Model file for the job. Use its own axes, mm. Face numbers are marked on the shaded views. A direction names the side the tool comes from. Round coordinates to 2 decimals unless told otherwise and drop trailing zeros. Loops run counter-clockwise (first coordinate to the right, second up) from the corner with the lowest first, then second, coordinate; pieces in that order, holes last. Notation, with made-up numbers: M 24,18.25 L 82,18.25 A14 cw 82,37.25 Z; hole C 61.25,35 d11. An arc over 180 degrees is marked long. Answer in a Markdown table with one row per item.
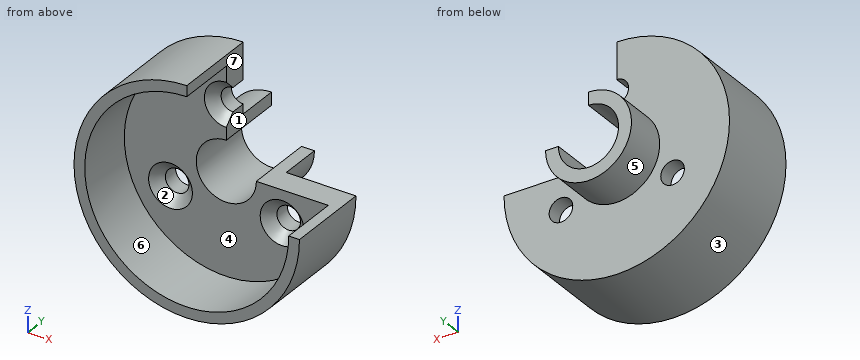
from build123d import *

# Parameters (mm, degrees)
COUNTERSUNK_HOLE_11_D             = 11
COUNTERSUNK_HOLE_11_CSINK_D       = 20.4
COUNTERSUNK_HOLE_11_CSINK_ANGLE   = 90
COUNTERSUNK_HOLE_PATTERN_3X_COUNT = 3
SIDE_SLOT_CUT_DEPTH               = 81.848623983
SIDE_SLOT_CUT_DEPTH_BACK          = 81.848623983


with BuildPart() as part:
    # Bed Profile Sketch → Bed Body Revolve (revolve)
    with BuildSketch(Plane(origin=(0, 0, 0), x_dir=(0, 0, -1), z_dir=(1, 0, 0))):
        Polygon((14, 30.393677345), (14, -1.606322655), (47.5, -1.606322655), (47.5, -29.606322655), (52.5, -29.606322655), (52.5, 10.393677345), (20, 10.393677345), (20, 30.393677345), align=None)
    revolve(axis=Axis((0, 0, 0), (0, 1, 0)))

    # Countersunk Hole Ø11 (through all)
    with Locations(Plane(origin=(0, -1.606322655, 30), x_dir=(0, 0, -1), z_dir=(0, -1, 0))):
        with Locations((0, 0)):
            countersunk_hole_11 = CounterSinkHole(COUNTERSUNK_HOLE_11_D / 2, COUNTERSUNK_HOLE_11_CSINK_D / 2, counter_sink_angle=COUNTERSUNK_HOLE_11_CSINK_ANGLE)

    # Countersunk Hole Pattern 3x: Countersunk Hole Ø11 ×3 about axis
    countersunk_hole_pattern_3x_axis = Axis((0, 0, 0), (0, 1, 0))
    for i in range(1, COUNTERSUNK_HOLE_PATTERN_3X_COUNT):
        add(countersunk_hole_11.rotate(countersunk_hole_pattern_3x_axis, i * 360 / COUNTERSUNK_HOLE_PATTERN_3X_COUNT), mode=Mode.SUBTRACT)

    # Side Slot Sketch → Side Slot Cut (cut, two sides: drawn at the far end of the back side and taken through both)
    with BuildSketch(Plane.XZ.offset(1.606322655).offset(-SIDE_SLOT_CUT_DEPTH_BACK)):
        with BuildLine():
            Line((0, 66.315052509), (0, 0))
            Line((0, 0), (70.372177226, 0))
            ThreePointArc((70.372177226, 0), (52.403266899, 51.428043669), (0, 66.315052509))
        make_face()
    extrude(amount=SIDE_SLOT_CUT_DEPTH + SIDE_SLOT_CUT_DEPTH_BACK, mode=Mode.SUBTRACT)


solid = part.part
1. Pin check, flat tips, straight feed: pin 1 (1 mm diameter, centred on x = 3.5, y = -16, fed in from +Z); pin 2 (4 mm diameter, centred on x = -36.5, z = 36, fed in from +Y); pin 3 (5 mm diameter, centred on x = -20, z = -37.5, fed in from -Y); pin 4 (9 mm diameter, centred on x = 25.98, z = -15, fed in from +Y). Stop position of each tip, or through.
Verdict:
| item | result |
|---|---|
| pin 1 | stops at z = -47.33 |
| pin 2 | stops at y = 10.39 |
| pin 3 | stops at y = -1.61 |
| pin 4 | passes through |
2. Saw through at A-A (z = 4). Write the cut outline in (x, y), and give its area (3 significant figures).
Verdict:
| item | result |
|---|---|
| outline | M -52.35,-29.61 L -47.33,-29.61 L -47.33,-1.61 L -13.42,-1.61 L -13.42,30.39 L -19.6,30.39 L -19.6,10.39 L -52.35,10.39 Z |
| area | 731 mm² |
3. Mould opens along X. For the marked faces 1, 2, 3 and 4 say: +X half, -X half, draft (parallel to the pull), parting line (faces both ways), or undercut.
Verdict:
| item | result |
|---|---|
| face 1 | +X half |
| face 2 | undercut |
| face 3 | parting line |
| face 4 | undercut |
4. Saw through at D-D (z = -45). Write the cut outline in (x, y), and give its area (3 significant figures).
Verdict:
| item | result |
|---|---|
| outline | M -27.04,-29.61 L -15.21,-29.61 L -15.21,-1.61 L 15.21,-1.61 L 15.21,-29.61 L 27.04,-29.61 L 27.04,10.39 L -27.04,10.39 Z |
| area | 1,310 mm² |
5. Saw through at C-C (x = 43.5). Write the cut outline in (y, z).
Verdict:
| item | result |
|---|---|
| outline | M -29.61,-29.39 L 10.39,-29.39 L 10.39,0 L -1.61,0 L -1.61,-19.08 L -29.61,-19.08 Z |
6. Saw through at B-B (y = 19.5). Write the cut outline in (x, z), and give its area (3 significant figures).
Verdict:
| item | result |
|---|---|
| outline | M 0,14 L 0,20 A20 ccw long 20,0 L 14,0 A14 cw long Z |
| area | 481 mm² |
7. Wall check: probe 1 along X at (y, z) = (8, -15); probe 2 along Y at (x, z) = (18, -24); probe 3 along Y at (x, z) = (-47, 23). Give the ranges that are in metal, low to high.
Verdict:
| item | result |
|---|---|
| probe 1 | x = -50.31 to -31.48, -20.48 to 20.48, 31.48 to 50.31 |
| probe 2 | y = -1.61 to 10.39 |
| probe 3 | y = -29.61 to 10.39 |
8. Tool access for the marked faces 5, 6 and 7: list every direction of +Z, -Z, +X, -X, +Y, -Y with a clear straight run to the whole face (end or side of a thin tool).
Verdict:
| item | result |
|---|---|
| face 5 | +Y |
| face 6 | -Y |
| face 7 | +Z, +X, +Y, -Y |
